Check sheet for the modelled part. Datum: model origin and axes. Units: mm. Round coordinates to 2 decimals unless told otherwise and drop trailing zeros. Order: outer loops, then holes, each group sorted by start corner. A loop starts at its lowest first (then second) coordinate and runs counter-clockwise, first axis right, second up.
Q1. Cross-section at B-B on x = -47.5. Record the cut outline in (y, z), then the cut area to 3 significant figures.
Q2. Cross-section at C-C on z = -0.7. Record the cut outline in (x, y).
Q3. Cross-section at A-A on y = 46. Record the cut outline in (x, z), then the cut area to 3 significant figures.
Q4. Cross-section at D-D on y = -48. Record the cut outline in (x, z).
Q5. Scan lines: probe 1 along Y at (x, z) = (-47.5, 1.55); probe 2 along X at (y, z) = (-46, 0.85); probe 3 along Y at (x, z) = (-46, 0). Record each from-to range of solid material in increasing order.
from build123d import *

# Parameters (mm, degrees)
SKETCH1_R           = 5.25
BOSS_EXTRUDE1_DEPTH = 3


with BuildPart() as part:
    # Sketch1 → Boss-Extrude1 (new, symmetric)
    with BuildSketch(Plane.XY):
        Polygon((-67.5, 60), (-62.5, 65), (62.5, 65), (67.5, 60), (67.5, -60), (62.5, -65), (-62.5, -65), (-67.5, -60), align=None)
        with Locations((-47.5, 46)):
            Circle(SKETCH1_R, mode=Mode.SUBTRACT)
        with Locations((-27.5, 46)):
            Circle(SKETCH1_R, mode=Mode.SUBTRACT)
        with Locations((44.5, 46)):
            Circle(SKETCH1_R, mode=Mode.SUBTRACT)
        with Locations(Location((44.5, -46, 0), (0, 0, 180))):
            Circle(SKETCH1_R, mode=Mode.SUBTRACT)
        with Locations(Location((-27.5, -46, 0), (0, 0, 180))):
            Circle(SKETCH1_R, mode=Mode.SUBTRACT)
        with Locations(Location((-47.5, -46, 0), (0, 0, 180))):
            Circle(SKETCH1_R, mode=Mode.SUBTRACT)
    extrude(amount=BOSS_EXTRUDE1_DEPTH, both=True)


solid = part.part
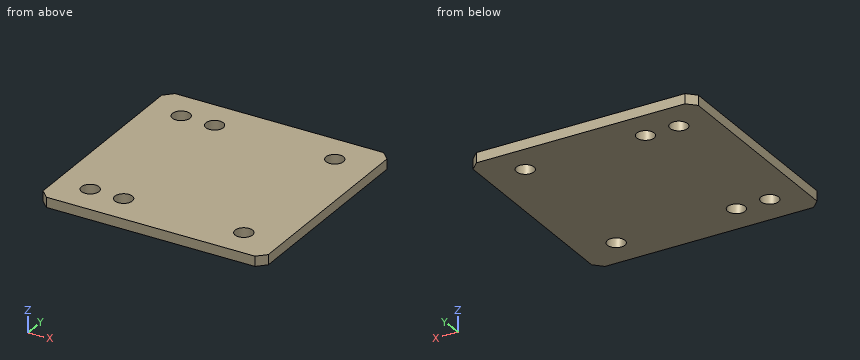
Results found:
1. outline: (-65, -3) - (-51.25, -3) - (-51.25, 3) - (-65, 3) - close; (-40.75, -3) - (40.75, -3) - (40.75, 3) - (-40.75, 3) - close; (51.25, -3) - (65, -3) - (65, 3) - (51.25, 3) - close
1. area: 654 mm2
2. outline: (-67.5, -60) - (-62.5, -65) - (62.5, -65) - (67.5, -60) - (67.5, 60) - (62.5, 65) - (-62.5, 65) - (-67.5, 60) - close; hole circle Ø10.5 at (-47.5, -46); hole circle Ø10.5 at (-47.5, 46); hole circle Ø10.5 at (-27.5, -46); hole circle Ø10.5 at (-27.5, 46); hole circle Ø10.5 at (44.5, -46); hole circle Ø10.5 at (44.5, 46)
3. outline: (-67.5, -3) - (-52.75, -3) - (-52.75, 3) - (-67.5, 3) - close; (-42.25, -3) - (-32.75, -3) - (-32.75, 3) - (-42.25, 3) - close; (-22.25, -3) - (39.25, -3) - (39.25, 3) - (-22.25, 3) - close; (49.75, -3) - (67.5, -3) - (67.5, 3) - (49.75, 3) - close
3. area: 621 mm2
4. outline: (-67.5, -3) - (-52.35, -3) - (-52.35, 3) - (-67.5, 3) - close; (-42.65, -3) - (-32.35, -3) - (-32.35, 3) - (-42.65, 3) - close; (-22.65, -3) - (39.65, -3) - (39.65, 3) - (-22.65, 3) - close; (49.35, -3) - (67.5, -3) - (67.5, 3) - (49.35, 3) - close
5. probe 1: y = -65 to -51.25, -40.75 to 40.75, 51.25 to 65
5. probe 2: x = -67.5 to -52.75, -42.25 to -32.75, -22.25 to 39.25, 49.75 to 67.5
5. probe 3: y = -65 to -51.03, -40.97 to 40.97, 51.03 to 65
